Here's the drawing with two shaded views (mm, measured from the low corner). I have some questions. Round coordinates to 2 decimals unless told otherwise and drop trailing zeros. Loops run counter-clockwise (first coordinate to the right, second up) from the corner with the lowest first, then second, coordinate; pieces in that order, holes last.
(1) If I drill on line 1 along X through (y, z) = (15, 6.75); line 2 along Y through (x, z) = (13, 3.25) (1 decimal); line 3 along Y through (x, z) = (17.5, 1.75) (1 decimal), over which ranges is the centre line in solid material (lowest first)?
(2) Thinking about a two-plate mould opening in Y: for the marked faces 1, 2, 3 and 4, which applies, released by +Y, released by -Y, zero draft, split by the parting line, or undercut?
(3) I want a section at B-B on z = 3. Write out the boundary of the cut face in (x, y), plus the area to 3 significant figures.
(4) Will these pins go through, and if not, where does the flat tip stop? pin 1 Ø12 at (x, y) = (21.5, 31) entering from +Z; pin 2 Ø1 at (y, z) = (27.5, 3) entering from -X (1 decimal); pin 3 Ø3 at (y, z) = (5, 3.5) entering from +X; pin 4 Ø4 at (y, z) = (30.5, 6.5) entering from +X (1 decimal).
(5) I want a section at A-A on z = 1. Write out the boundary of the cut face in (x, y) (1 decimal).
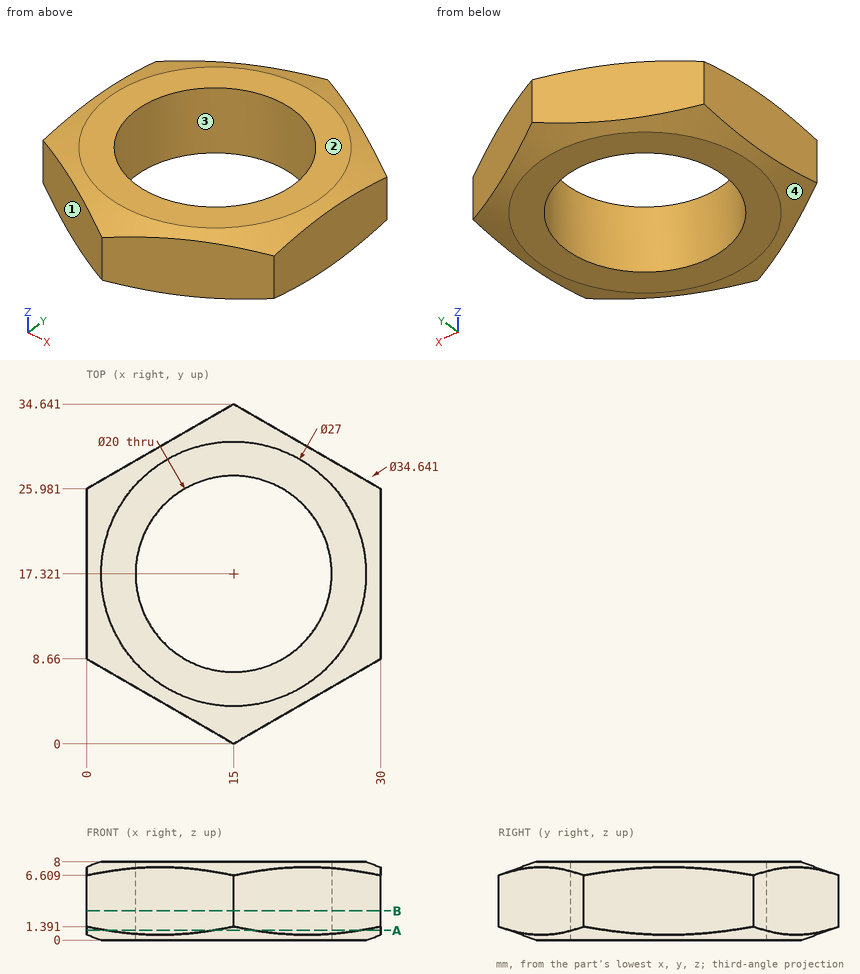
Filled sheet:
1. line 1: x = 0 to 5.27, 24.73 to 30
1. line 2: y = 1.2 to 7.5, 27.1 to 33.5
1. line 3: y = 1.4 to 7.6, 27 to 33.2
2. face 1: released by -Y
2. face 2: zero draft
2. face 3: undercut
2. face 4: split by the parting line
3. outline: (0, 8.66) - (15, 0) - (30, 8.66) - (30, 25.98) - (15, 34.64) - (0, 25.98) - close; hole circle Ø20 at (15, 17.32)
3. area: 465 mm2
4. pin 1: stops at z = 8
4. pin 2: stops at x = 1.8
4. pin 3: stops at x = 26.26
4. pin 4: stops at x = 25.6
5. outline: (0, 11.1) arc R16.2 ccw to (2.1, 7.5) - (12.9, 1.2) arc R16.2 ccw to (17.1, 1.2) - (27.9, 7.5) arc R16.2 ccw to (30, 11.1) - (30, 23.6) arc R16.2 ccw to (27.9, 27.2) - (17.1, 33.4) arc R16.2 ccw to (12.9, 33.4) - (2.1, 27.2) arc R16.2 ccw to (0, 23.6) - close; hole circle Ø20 at (15, 17.3)
